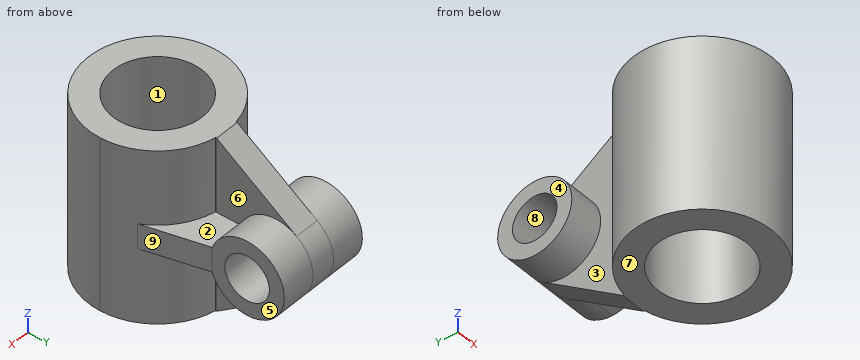
```python
from build123d import *

# Parameters (mm, degrees)
MAIN_CYLINDER_SKETCH_R = 14
MAIN_CYLINDER_28_DEPTH = 35
MAIN_BORE_SKETCH_R     = 9
MAIN_BORE_18_DEPTH     = 35
BASE_WEB_SKETCH_R      = 7.5
BASE_WEB_DEPTH         = 2.5
SECOND_WEB_DEPTH       = 2.5
SUPPORT_RIB_DEPTH      = 5
UPPER_BOSS_A_SKETCH_R  = 7.5
UPPER_BOSS_A_15_DEPTH  = 7
UPPER_BOSS_B_SKETCH_R  = 7.5
UPPER_BOSS_B_15_DEPTH  = 7
BOSS_ARM_DEPTH         = 7
SADDLE_FILL_DEPTH      = 35
TRIM_CUT_1_DEPTH       = 15
TRIM_CUT_2_DEPTH       = 51.430645445
TRIM_CUT_2_DEPTH_BACK  = 15
TRIM_CUT_3_DEPTH       = 15
UPPER_BORE_SKETCH_R    = 4.5
UPPER_BORE_9_DEPTH     = 50
CYLINDER_SKIN_28_DEPTH = 35


with BuildPart() as part:
    # Main Cylinder Sketch → Main Cylinder _28 (new body)
    with BuildSketch(Plane.XY):
        Circle(MAIN_CYLINDER_SKETCH_R)
    extrude(amount=-MAIN_CYLINDER_28_DEPTH)

    # Main Bore Sketch → Main Bore _18 (cut)
    with BuildSketch(Plane.XY):
        Circle(MAIN_BORE_SKETCH_R)
    extrude(amount=-MAIN_BORE_18_DEPTH, mode=Mode.SUBTRACT)



with BuildPart() as body_2:
    # Base Web Sketch → Base Web (new body)
    with BuildSketch(Plane(origin=(0, 0, 0), x_dir=(0, 0, -1), z_dir=(1, 0, 0))):
        with Locations((17.5, 26)):
            Circle(BASE_WEB_SKETCH_R)
        with BuildLine():
            Line((35, 14), (25, 26))
            ThreePointArc((25, 26), (17.5, 18.5), (10, 26))
            Line((10, 26), (0, 14))
            Line((0, 14), (35, 14))
        make_face()
    extrude(amount=-BASE_WEB_DEPTH)

    # Second Web Sketch → Second Web (add)
    with BuildSketch(Plane(origin=(0, 0, 0), x_dir=(0, 0, -1), z_dir=(1, 0, 0))):
        with BuildLine():
            ThreePointArc((25, 26), (17.5, 33.5), (10, 26))
            ThreePointArc((10, 26), (17.5, 18.5), (25, 26))
        make_face()
        with BuildLine():
            Line((10, 26), (0, 14))
            Line((0, 14), (35, 14))
            Line((35, 14), (25, 26))
            ThreePointArc((25, 26), (17.5, 18.5), (10, 26))
        make_face()
    extrude(amount=SECOND_WEB_DEPTH)

    # Support Rib Sketch → Support Rib (add)
    with BuildSketch(Plane(origin=(2.5, 0, 0), x_dir=(0, 0, -1), z_dir=(1, 0, 0))):
        with BuildLine():
            Line((11.267674623, 30.172303968), (0, 14))
            Line((0, 14), (10, 26))
            ThreePointArc((10, 26), (10.323913311, 28.180316454), (11.267674623, 30.172303968))
        make_face()
        with BuildLine():
            Line((25, 26), (35, 14))
            Line((35, 14), (23.732325377, 30.172303968))
            ThreePointArc((23.732325377, 30.172303968), (24.676086689, 28.180316454), (25, 26))
        make_face()
    extrude(amount=-SUPPORT_RIB_DEPTH)

    # Upper Boss A Sketch → Upper Boss A _15 (add)
    with BuildSketch(Plane(origin=(2.5, 0, 0), x_dir=(0, 0, -1), z_dir=(1, 0, 0))):
        with Locations((17.5, 26)):
            Circle(UPPER_BOSS_A_SKETCH_R)
    extrude(amount=UPPER_BOSS_A_15_DEPTH)

    # Upper Boss B Sketch → Upper Boss B _15 (add)
    with BuildSketch(Plane.ZY.offset(2.5)):
        with Locations(Location((-17.5, 26, 0), (0, 0, 180))):
            Circle(UPPER_BOSS_B_SKETCH_R)
    extrude(amount=UPPER_BOSS_B_15_DEPTH)

    # Upper Bore Sketch → Upper Bore _9 (cut)
    with BuildSketch(Plane(origin=(9.5, 0, 0), x_dir=(0, 0, -1), z_dir=(1, 0, 0))):
        with Locations((17.5, 26)):
            Circle(UPPER_BORE_SKETCH_R)
    extrude(amount=-UPPER_BORE_9_DEPTH, mode=Mode.SUBTRACT)


with BuildPart() as body_3:
    # Boss Arm Sketch → Boss Arm (new body)
    with BuildSketch(Plane(origin=(9.5, 0, 0), x_dir=(0, 0, -1), z_dir=(1, 0, 0))):
        with BuildLine():
            Line((15, 18.5), (15, 18.928932188))
            ThreePointArc((15, 18.928932188), (17.5, 18.5), (20, 18.928932188))
            Line((20, 18.928932188), (20, 0))
            Line((20, 0), (15, 0))
            Line((15, 0), (15, 18.5))
        make_face()
    extrude(amount=-BOSS_ARM_DEPTH)

    # Trim Cut 3 Sketch → Trim Cut 3 (cut)
    with BuildSketch(Plane.XY.offset(-15)):
        with BuildLine():
            Line((2.5, 0), (9, 0))
            ThreePointArc((9, 0), (7.193747285, 5.408326913), (2.5, 8.645808233))
            Line((2.5, 8.645808233), (2.5, 0))
        make_face()
    extrude(amount=-TRIM_CUT_3_DEPTH, mode=Mode.SUBTRACT)


with BuildPart() as body_4:
    # Saddle Fill Sketch → Saddle Fill (new body)
    with BuildSketch(Plane.XY):
        with BuildLine():
            Line((9.5, 18.928932188), (12.50219707, 6.300402243))
            ThreePointArc((12.50219707, 6.300402243), (8.380560683, 11.214553163), (2.5, 13.774977314))
            Line((2.5, 13.774977314), (2.5, 18.928932188))
            Line((2.5, 18.928932188), (9.5, 18.928932188))
        make_face()
    extrude(amount=-SADDLE_FILL_DEPTH)

    # Trim Cut 1 Sketch → Trim Cut 1 (cut)
    with BuildSketch(Plane.XY):
        with BuildLine():
            Line((2.5, 18.928932188), (9.5, 18.928932188))
            Line((9.5, 18.928932188), (12.50219707, 6.300402243))
            ThreePointArc((12.50219707, 6.300402243), (8.380560683, 11.214553163), (2.5, 13.774977314))
            Line((2.5, 13.774977314), (2.5, 18.928932188))
        make_face()
    extrude(amount=-TRIM_CUT_1_DEPTH, mode=Mode.SUBTRACT)

    # Trim Cut 2 Sketch → Trim Cut 2 (cut, two sides: drawn at the far end of the back side and taken through both)
    with BuildSketch(Plane(origin=(0, 0, -35), x_dir=(-1, 0, 0), z_dir=(0, 0, -1)).offset(-TRIM_CUT_2_DEPTH_BACK)):
        with BuildLine():
            Line((-2.5, 18.928932188), (-9.5, 18.928932188))
            Line((-9.5, 18.928932188), (-12.50219707, 6.300402243))
            ThreePointArc((-12.50219707, 6.300402243), (-8.380560683, 11.214553163), (-2.5, 13.774977314))
            Line((-2.5, 13.774977314), (-2.5, 18.928932188))
        make_face()
    extrude(amount=TRIM_CUT_2_DEPTH + TRIM_CUT_2_DEPTH_BACK, mode=Mode.SUBTRACT)


with BuildPart() as part_1:
    add(part.part)

    add(body_2.part)  # Cylinder Skin _28 merges body 2

    add(body_3.part)  # Cylinder Skin _28 merges body 3

    add(body_4.part)  # Cylinder Skin _28 merges body 4
    # Cylinder Skin Sketch → Cylinder Skin _28 (add)
    with BuildSketch(Plane.XY):
        with BuildLine():
            Line((2.5, 14), (1.6e-08, 14))
            ThreePointArc((1.6e-08, 14), (1.252779423, 13.94383533), (2.495507125, 13.775791962))
            Line((2.495507125, 13.775791962), (2.5, 14))
        make_face()
        with BuildLine():
            Line((1.6e-08, 14), (-2.5, 14))
            Line((-2.5, 14), (-2.5, 13.774977314))
            ThreePointArc((-2.5, 13.774977314), (-1.255053299, 13.943630848), (1.6e-08, 14))
        make_face()
    extrude(amount=-CYLINDER_SKIN_28_DEPTH)


solid = part_1.part
```
Geometry: final body of the model. Coordinates: model frame, mm. Face numbers are marked on the shaded views. A direction names the side the tool comes from. Coordinates: 2 decimals unless noted, no trailing zeros. Order: outer loops, then holes, each group sorted by start corner. A loop starts at its lowest first (then second) coordinate and runs counter-clockwise, first axis right, second up. Notation, with made-up numbers: (35.25, 87.25) - (85.25, 87.25) arc R17 ccw to (85.25, 112.25) - close; hole circle Ø6 at (61.25, -19.75). An arc over 180 degrees is marked (long way). Return JSON: item names as keys, results as strings. Group by question number.
1. Cut plane A-A (x = 0). Output: boundary loops of the cut face in (y, z), plus the area to 3 significant figures.
2. Cut plane D-D (z = -23). Output: boundary loops of the cut face in (x, y).
3. Pin query (flat end, axial travel): pin 1 (8 mm diameter, centred on y = 23.5, z = -20.5, fed in from -X); pin 2 (5 mm diameter, centred on y = -8.5, z = -4.5, fed in from +X); pin 3 (4 mm diameter, centred on y = 26, z = -6.5, fed in from +X); pin 4 (11 mm diameter, centred on x = 5.5, y = 14, fed in from +Z). Return the tip coordinate at first contact, or that it passes through.
4. Cut plane B-B (z = -16.5). Count the separate pieces of the cut face and the enclosed holes in it, plus the area to 3 significant figures.
5. Set-up query: the marked faces 1, 2, 3, 4 and 5. Return all of +Z, -Z, +X, -X, +Y, -Y with unobstructed straight access to the full face (end or side cutting, diameter ignored); none if empty.
6. Material intervals for line 1 along Y through (x, z) = (0, -11.5); line 2 along Y through (x, z) = (0, -17.5); line 3 along Y through (x, z) = (-2.25, -17.5), sorted ascending. Write a range as [from, to].
7. Pull-direction query (Y, two-part tool) for the marked faces 6, 7, 8 and 9; classes: pulls with the +Y half, pulls with the -Y half, needs draft (parallel to the pull), parting line crosses it, or undercut.
8. Cut plane C-C (x = -7.25). Output: boundary loops of the cut face in (y, z), plus the area to 3 significant figures.
Resolved:
{
 "1": {"outline": "(-14, -35) - (-9, -35) - (-9, 0) - (-14, 0) - close; (9, -35) - (14, -35) - (30.17, -23.73) arc R7.5 ccw to (30.17, -11.27) - (14, 0) - (9, 0) - close; hole circle Ø9 at (26, -17.5)", "area": "699 mm²"},
 "2": {"outline": "(-9.5, 20.9) - (-2.5, 20.9) - (-2.5, 13.77) arc R14 ccw (long way) to (2.5, 13.78) - (2.5, 14) - (2.5, 20.9) - (9.5, 20.9) - (9.5, 31.1) - (-9.5, 31.1) - close; hole circle Ø18 at (0, 0)"},
 "3": {"pin 1": "stops at x = -9.5", "pin 2": "stops at x = 12.65", "pin 3": "stops at x = 2.5", "pin 4": "stops at z = 0"},
 "4": {"separate pieces": "2", "enclosed holes": "2", "area": "555 mm²"},
 "5": {"face 1": "+Z, -Z", "face 2": "+Z, +X", "face 3": "-X", "face 4": "+Z, -Z, -X, +Y", "face 5": "+Z, -Z, +X, +Y"},
 "6": {"line 1": "y = [-14, -9], [9, 30.5]", "line 2": "y = [-14, -9], [9, 21.5], [30.5, 33.5]", "line 3": "y = [-13.82, -8.71], [8.71, 21.5], [30.5, 33.5]"},
 "7": {"face 6": "undercut", "face 7": "needs draft", "face 8": "undercut", "face 9": "pulls with the +Y half"},
 "8": {"outline": "(-11.98, -35) - (-5.33, -35) - (-5.33, 0) - (-11.98, 0) - close; (5.33, -35) - (11.98, -35) - (11.98, 0) - (5.33, 0) - close; circle Ø15 at (26, -17.5); hole circle Ø9 at (26, -17.5)", "area": "578 mm²"}
}
